Build history of the part. All positions in model axes, mm. Face numbers are marked on the shaded views. Coordinates: 2 decimals unless noted, no trailing zeros. Loops run counter-clockwise (first coordinate to the right, second up) from the corner with the lowest first, then second, coordinate; pieces in that order, holes last.
(1) Slice it at B-B (x = -3). Give the cut face in (y, z), and give its area (3 significant figures).
(2) Two-plate mould, pull along Z, no slides. Class the marked faces 1, 2 and 3: pulls with the +Z half, pulls with the -Z half, needs draft (parallel to the pull), parting line crosses it, or undercut.
(3) Wall check: L1, parallel to X at y = 23, z = 213; L2, parallel to X at y = 5.5, z = 113; L3, parallel to Y at x = -0.5, z = 218. Give the ranges that are in metal, low to high.
(4) Flat gauge pins, fed straight in: P1, Ø12, axis at x = 6.5, z = 47, coming from the +Y side; P2, Ø4.5, axis at y = 5.5, z = 108, coming from the +X side; P3, Ø10, axis at y = 21.5, z = 178.5, coming from the -X side. Where does each tip first touch, or does it go through?
(5) Slice it at A-A (y = 30). Give the cut face in (x, z).
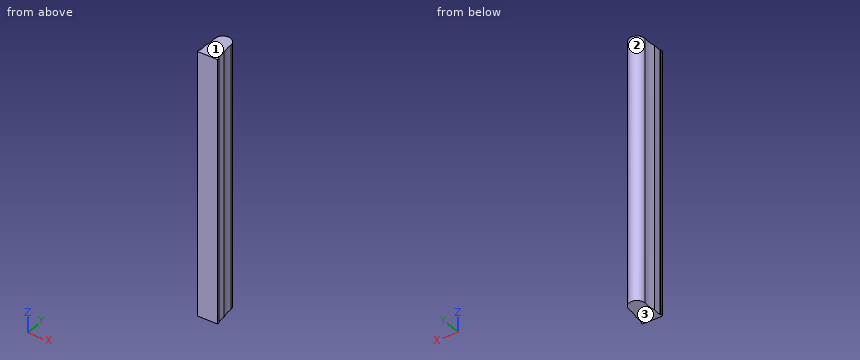
from build123d import *

# Parameters (mm, degrees)
EXTRUDE_1_DEPTH = 300


with BuildPart() as part:
    # 草图1 → 凸台-拉伸1 (new body)
    with BuildSketch(Plane.XY):
        with BuildLine():
            Line((10, 12), (10, 2.8))
            Line((10, 2.8), (11, 2.8))
            Line((11, 2.8), (11, 0))
            Line((11, 0), (-11, 0))
            Line((-11, 0), (-11, 2.8))
            Line((-11, 2.8), (-10, 2.8))
            Line((-10, 2.8), (-10, 12))
            add(Edge.make_bspline(
                [(-8.8, 25.2), (-8.148207528, 18.483731085), (-10, 12)],
                knots=[0, 0, 0, 1, 1, 1], degree=2))
            ThreePointArc((-8.8, 25.2), (0, 34), (8.8, 25.2))
            add(Edge.make_bspline(
                [(8.8, 25.2), (8.148207528, 18.483731085), (10, 12)],
                knots=[0, 0, 0, 1, 1, 1], degree=2))
        make_face()
    extrude(amount=EXTRUDE_1_DEPTH)


solid = part.part
Response values:
1. outline: (0, 0) - (33.47, 0) - (33.47, 300) - (0, 300) - close
1. area: 10,000 mm2
2. face 1: pulls with the +Z half
2. face 2: needs draft
2. face 3: pulls with the -Z half
3. L1: x = -8.65 to 8.65
3. L2: x = -10 to 10
3. L3: y = 0 to 33.99
4. P1: stops at y = 33.99
4. P2: stops at x = 10
4. P3: stops at x = -9.02
5. outline: (-7.38, 0) - (7.38, 0) - (7.38, 300) - (-7.38, 300) - close
